Study the drawing (mm; zero at the part's minimum x, y, z) and answer. A direction names the side the tool comes from. Round coordinates to 2 decimals unless told otherwise and drop trailing zeros. Write each loop counter-clockwise with the first axis right and the second up, starting at its lowest first coordinate (ties: lowest second). Pieces come first, ordered by that corner, then holes. Notation, with made-up numbers: (87.25, 16.25) -> (114.25, 16.25) arc R17 ccw to (114.25, 47.25) -> close; hole circle Ø8 at (-21.5, 50.5). An arc over 180 degrees is marked (long way). Return JSON: item names as keys, results as strings.
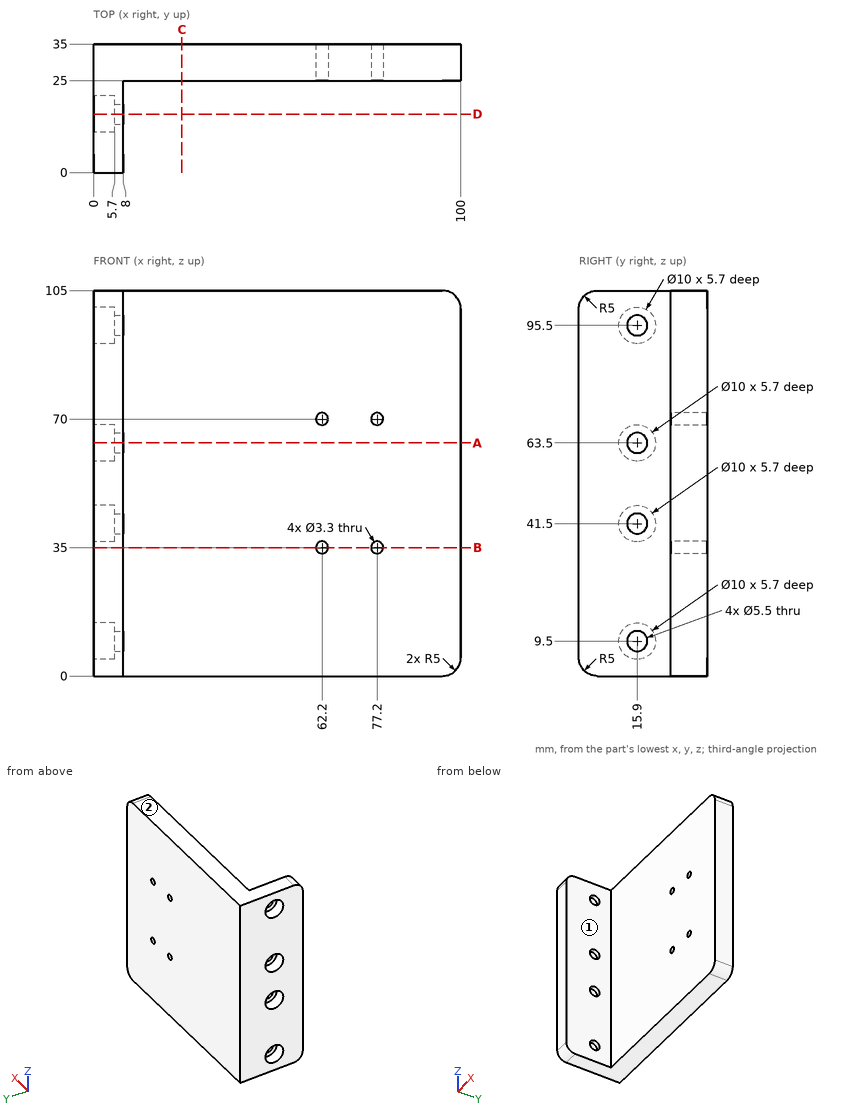
Item 1: Section D-D (y = 15.9) is taken. State how many separate pieces and enclosed holes the cut face has, then the cut area to 3 significant figures.
Worked answers:
{"separate pieces": "5", "enclosed holes": "0", "area": "561 mm2"}
Item 2: Section B-B (z = 35) is taken. Give the vertices of the cut face in (x, y), then the cut area to 3 significant figures.
Worked answers:
{"outline": "(0, 0) -> (8, 0) -> (8, 25) -> (60.55, 25) -> (60.55, 35) -> (0, 35) -> close; (63.85, 25) -> (75.55, 25) -> (75.55, 35) -> (63.85, 35) -> close; (78.85, 25) -> (100, 25) -> (100, 35) -> (78.85, 35) -> close", "area": "1,130 mm2"}
Item 3: Section C-C (x = 24) is taken. Give the vertices of the cut face in (y, z), then the cut area to 3 significant figures.
Worked answers:
{"outline": "(25, 0) -> (35, 0) -> (35, 105) -> (25, 105) -> close", "area": "1,050 mm2"}
Item 4: A tool of negligible diameter and unlimited length cuts with its end or side. For the marked faces 1 and 2, from which of +Z, -Z, +X, -X, +Y, -Y can it reach the whole face along a straight path? Write none if from no direction.
Worked answers:
{"face 1": "+Z, -Z, +X, -Y", "face 2": "+Z, +X, -X, +Y, -Y"}
Item 5: Straight lines are drawn through the part: L1, parallel to Z at x = 77.2, y = 32.5; L2, parallel to Z at x = 1.5, y = 15.9; L3, parallel to Y at x = 4.2, z = 41.5. For each, find the intervals that lie inside material, in ascending order. Write a range as [from, to].
Worked answers:
{"L1": "z = [0, 33.35], [36.65, 68.35], [71.65, 105]", "L2": "z = [0, 4.5], [14.5, 36.5], [46.5, 58.5], [68.5, 90.5], [100.5, 105]", "L3": "y = [0, 10.9], [20.9, 35]"}
Item 6: Section A-A (z = 63.5) is taken. Give the vertices of the cut face in (x, y), then the cut area to 3 significant figures.
Worked answers:
{"outline": "(0, 0) -> (8, 0) -> (8, 13.15) -> (5.7, 13.15) -> (5.7, 10.9) -> (0, 10.9) -> close; (0, 20.9) -> (5.7, 20.9) -> (5.7, 18.65) -> (8, 18.65) -> (8, 25) -> (100, 25) -> (100, 35) -> (0, 35) -> close", "area": "1,130 mm2"}
Item 7: Flat-ended cylindrical pins translate along their axes: pin 1 (5 mm diameter, centred on y = 16.5, z = 62, fed in from -X); pin 2 (2.5 mm diameter, centred on x = 62.2, z = 70, fed in from -Y); pin 3 (13 mm diameter, centred on y = 15.9, z = 9.5, fed in from +X); pin 4 (5.5 mm diameter, centred on x = 77.2, z = 35, fed in from -Y). Find the tip coordinate at first contact, or state that the pin passes through.
Worked answers:
{"pin 1": "stops at x = 5.7", "pin 2": "passes through", "pin 3": "stops at x = 8", "pin 4": "stops at y = 25"}
